Design review of the part shown in the three views and the two pictorial views. Dimensions are in mm from the part's minimum x, y and z. A direction names the side the tool comes from. Coordinates: 2 decimals unless noted, no trailing zeros. Loops run counter-clockwise (first coordinate to the right, second up) from the corner with the lowest first, then second, coordinate; pieces in that order, holes last. Notation, with made-up numbers: M -27.75,-16 L -21.75,-16 A29 cw -21.75,23 Z; hole C 74.25,0.25 d3. An arc over 180 degrees is marked long. Use CSV: the item, a comma, the result in double quotes. Start each with the question number.
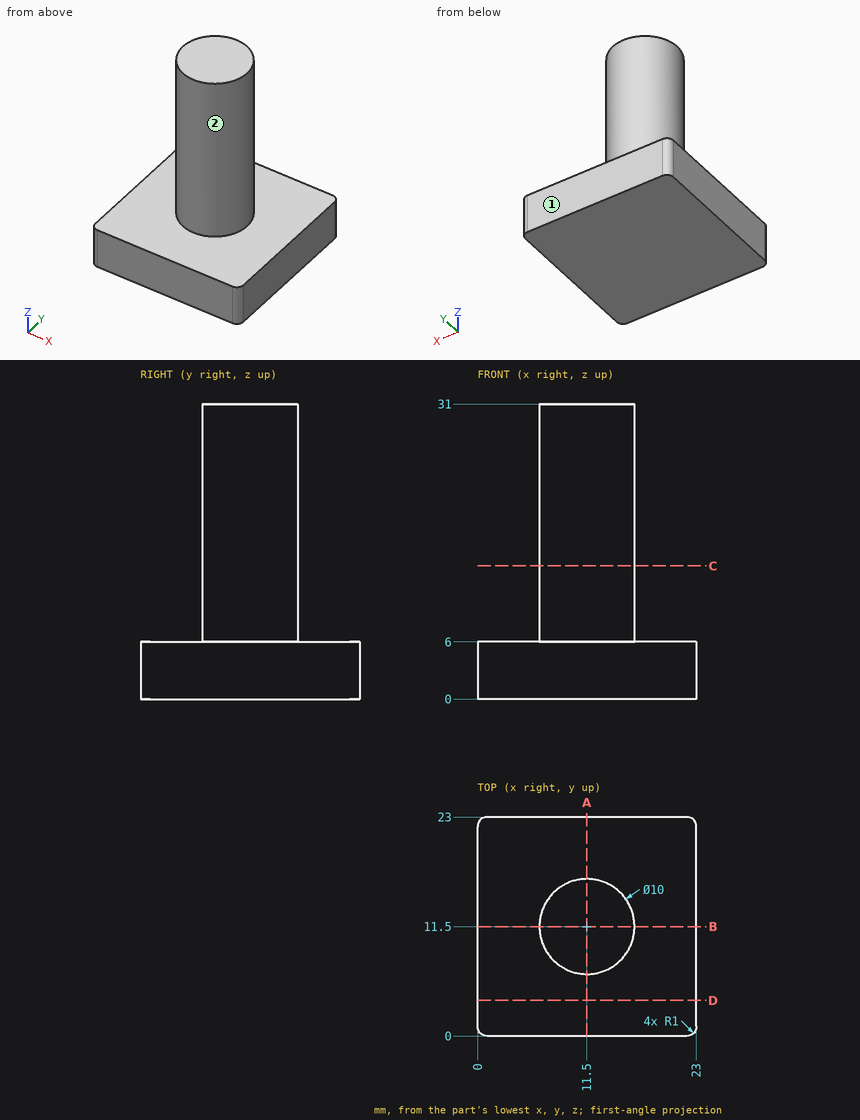
1. Add section A-A (x = 11.5). Write out the cut boundary in (y, z), plus the area to 3 significant figures.
2. For the marked faces 1 and 2, list the 3-axis set-ups (+Z, -Z, +X, -X, +Y, -Y) from which the entire face can be reached by the end or side of a thin tool; tool diameter is ignored.
3. Add section C-C (z = 14). Write out the cut boundary in (x, y).
4. Insertion check: pin 1 Ø1.5 at (y, z) = (17.5, 11.5) entering from +X; pin 2 Ø8 at (x, z) = (13.5, 19) entering from -Y; pin 3 Ø2 at (x, z) = (8, 12) entering from -Y; pin 4 Ø8 at (x, z) = (7.5, 25.5) entering from +Y. Each pin has a flat end and moves straight along its axis. Give the tip position at first contact, or say it passes through.
5. Add section D-D (y = 3.75). Write out the cut boundary in (x, z), plus the area to 3 significant figures.
6. To check wall thickness, follow line 1 along Z through (x, y) = (2, 12.5); line 2 along Y through (x, z) = (8.5, 27); line 3 along X through (y, z) = (14.75, 24). State the ranges of each line that lie inside material, in increasing order.
Solved:
1,outline,"M 0,0 L 23,0 L 23,6 L 16.5,6 L 16.5,31 L 6.5,31 L 6.5,6 L 0,6 Z"
1,area,"388 mm^2"
2,face 1,"+Z, -Z, +X, -X, +Y"
2,face 2,"+Z"
3,outline,"C 11.5,11.5 d10"
4,pin 1,"passes through"
4,pin 2,"stops at y = 6.5"
4,pin 3,"stops at y = 7.17"
4,pin 4,"stops at y = 16.5"
5,outline,"M 0,0 L 23,0 L 23,6 L 0,6 Z"
5,area,"138 mm^2"
6,line 1,"z = 0 to 6"
6,line 2,"y = 7.5 to 15.5"
6,line 3,"x = 7.7 to 15.3"
